Could you check a few things on this model? Use its own coordinates, in mm. Give positions to 0.01 mm unless a question says otherwise; leave off trailing zeros. Loops run counter-clockwise (first coordinate to the right, second up) from the corner with the lowest first, then second, coordinate; pieces in that order, holes last. Notation, with made-up numbers: (35, 57.25) -> (40, 57.25) arc R35 ccw to (40, 89.25) -> close; hole circle Ø6 at (54, 25.25). An arc over 180 degrees is marked (long way). Put each result on its own line as item: value.
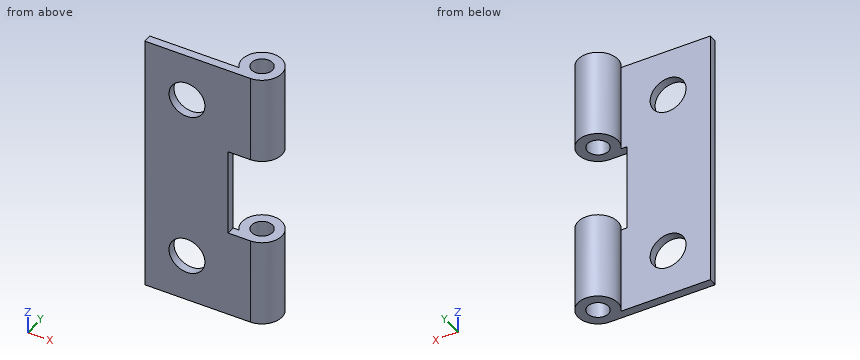
```python
from build123d import *

# Parameters (mm, degrees)
SKETCH_1_R          = 1
EXTRUDE_1_DEPTH     = 25
CUT_EXTRUDE_1_DEPTH = 3.8
SKETCH_3_R          = 1.7
CUT_EXTRUDE_2_DEPTH = 0.8
SKETCH_4_R          = 1.7
CUT_EXTRUDE_3_DEPTH = 0.8


with BuildPart() as part:
    # 草图1 → 凸台-拉伸1 (new body)
    with BuildSketch(Plane.XY):
        with BuildLine():
            Line((-10, 0), (0, 0))
            ThreePointArc((0, 0), (0.871779789, 3.588194302), (-1.549193338, 0.8))
            Line((-1.549193338, 0.8), (-10, 0.8))
            Line((-10, 0.8), (-10, 0))
        make_face()
        with Locations((0, 1.9)):
            Circle(SKETCH_1_R, mode=Mode.SUBTRACT)
    extrude(amount=-EXTRUDE_1_DEPTH)

    # 草图2 → 切除-拉伸1 (cut)
    with BuildSketch(Plane(origin=(0, 0, 0), x_dir=(1, 0, 0), z_dir=(0, 1, 0))):
        Polygon((-2.09, 8.333333333), (2.09, 8.333333333), (2.09, 0), (6, 0), (6, 25), (2.09, 25), (2.09, 16.666666667), (-2.09, 16.666666667), align=None)
    extrude(amount=CUT_EXTRUDE_1_DEPTH, mode=Mode.SUBTRACT)

    # 草图3 → 切除-拉伸2 (cut)
    with BuildSketch(Plane(origin=(0, 0, 0), x_dir=(1, 0, 0), z_dir=(0, 1, 0))):
        with Locations(Location((-6, 20.5, 0), (0, 0, 270))):
            Circle(SKETCH_3_R)
    extrude(amount=CUT_EXTRUDE_2_DEPTH, mode=Mode.SUBTRACT)

    # 草图4 → 切除-拉伸3 (cut)
    with BuildSketch(Plane(origin=(0, 0, 0), x_dir=(1, 0, 0), z_dir=(0, 1, 0))):
        with Locations(Location((-6, 4.5, 0), (0, 0, 270))):
            Circle(SKETCH_4_R)
    extrude(amount=CUT_EXTRUDE_3_DEPTH, mode=Mode.SUBTRACT)


solid = part.part
```
1. If we section it at B-B (y = 1.9): List the corners of the cut face in (x, z) for me.
Recorded:
outline: (-1.9, -25) -> (-1, -25) -> (-1, -16.67) -> (-1.9, -16.67) -> close; (-1.9, -8.33) -> (-1, -8.33) -> (-1, 0) -> (-1.9, 0) -> close; (1, -25) -> (1.9, -25) -> (1.9, -16.67) -> (1, -16.67) -> close; (1, -8.33) -> (1.9, -8.33) -> (1.9, 0) -> (1, 0) -> close
2. If we section it at A-A (z = -4.5): List the corners of the cut face in (x, y) for me, then the cut area to 3 significant figures.
Recorded:
outline: (-10, 0) -> (-7.7, 0) -> (-7.7, 0.8) -> (-10, 0.8) -> close; (-4.3, 0) -> (0, 0) arc R1.9 ccw (long way) to (-1.55, 0.8) -> (-4.3, 0.8) -> close; hole circle Ø2 at (0, 1.9)
area: 12.6 mm^2
3. If we section it at D-D (x = -6): List the corners of the cut face in (y, z) for me, then the cut area to 3 significant figures.
Recorded:
outline: (0, -25) -> (0.8, -25) -> (0.8, -22.2) -> (0, -22.2) -> close; (0, -18.8) -> (0.8, -18.8) -> (0.8, -6.2) -> (0, -6.2) -> close; (0, -2.8) -> (0.8, -2.8) -> (0.8, 0) -> (0, 0) -> close
area: 14.6 mm^2
4. If we section it at C-C (x = 0.25): List the corners of the cut face in (y, z) for me, then the cut area to 3 significant figures.
Recorded:
outline: (0.02, -25) -> (0.93, -25) -> (0.93, -16.67) -> (0.02, -16.67) -> close; (0.02, -8.33) -> (0.93, -8.33) -> (0.93, 0) -> (0.02, 0) -> close; (2.87, -25) -> (3.78, -25) -> (3.78, -16.67) -> (2.87, -16.67) -> close; (2.87, -8.33) -> (3.78, -8.33) -> (3.78, 0) -> (2.87, 0) -> close
area: 30.5 mm^2
5. I'm going to push flat-ended pins straight in: pin 1 (1 mm diameter, centred on y = 0.5, z = -17, fed in from +X); pin 2 (4 mm diameter, centred on x = -6, z = -6.5, fed in from +Y); pin 3 (0.9 mm diameter, centred on y = 0.5, z = -12, fed in from +X). Where does each tip first touch, or does it pass through?
Recorded:
pin 1: stops at x = 1.67
pin 2: stops at y = 0.8
pin 3: stops at x = -2.09
6. I need wall thicknesses on line 1 (Z direction, x = 1.25, y = 1.1); line 2 (Y direction, x = -5.5, z = -7); line 3 (X direction, y = 0.3, z = -20.5). Which ranges of each line are inside material? Lowest first, please.
Recorded:
line 1: z = -25 to -16.67, -8.33 to 0
line 2: y = 0 to 0.8
line 3: x = -10 to -7.7, -4.3 to 1.02
